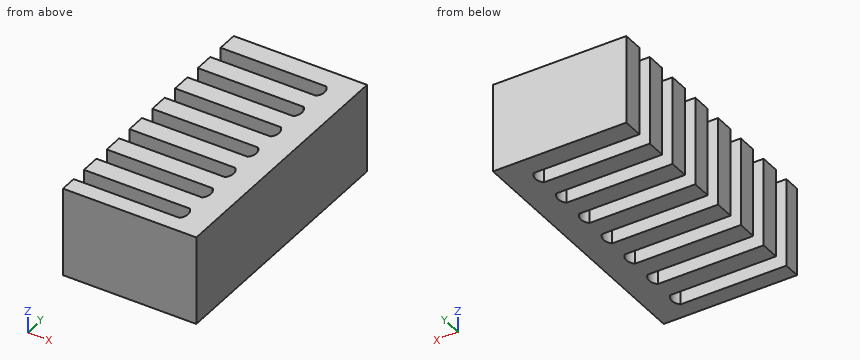
from build123d import *

# Parameters (mm, degrees)
EXTRUDE_1_DEPTH = 5


with BuildPart() as part:
    # 草图1 → 凸台-拉伸1 (new, symmetric)
    with BuildSketch(Plane.XY):
        with BuildLine():
            Line((7.5, -15), (-7.5, -15))
            Line((-7.5, -15), (-7.5, -13.125870379))
            Line((-7.5, -13.125870379), (4.407309833, -13.125870379))
            ThreePointArc((4.407309833, -13.125870379), (4.784555906, -12.215117792), (4.407309833, -11.304365204))
            Line((4.407309833, -11.304365204), (-7.5, -11.304365204))
            Line((-7.5, -11.304365204), (-7.5, -9.125870379))
            Line((-7.5, -9.125870379), (4.407309833, -9.125870379))
            ThreePointArc((4.407309833, -9.125870379), (4.784555906, -8.215117792), (4.407309833, -7.304365204))
            Line((4.407309833, -7.304365204), (-7.5, -7.304365204))
            Line((-7.5, -7.304365204), (-7.5, -5.125870379))
            Line((-7.5, -5.125870379), (4.407309833, -5.125870379))
            ThreePointArc((4.407309833, -5.125870379), (4.784555906, -4.215117792), (4.407309833, -3.304365204))
            Line((4.407309833, -3.304365204), (-7.5, -3.304365204))
            Line((-7.5, -3.304365204), (-7.5, -1.125870379))
            Line((-7.5, -1.125870379), (4.407309833, -1.125870379))
            ThreePointArc((4.407309833, -1.125870379), (4.784555906, -0.215117792), (4.407309833, 0.695634796))
            Line((4.407309833, 0.695634796), (-7.5, 0.695634796))
            Line((-7.5, 0.695634796), (-7.5, 2.874129621))
            Line((-7.5, 2.874129621), (4.407309833, 2.874129621))
            ThreePointArc((4.407309833, 2.874129621), (4.784555906, 3.784882208), (4.407309833, 4.695634796))
            Line((4.407309833, 4.695634796), (-7.5, 4.695634796))
            Line((-7.5, 4.695634796), (-7.5, 6.874129621))
            Line((-7.5, 6.874129621), (4.407309833, 6.874129621))
            ThreePointArc((4.407309833, 6.874129621), (4.784555906, 7.784882208), (4.407309833, 8.695634796))
            Line((4.407309833, 8.695634796), (-7.5, 8.695634796))
            Line((-7.5, 8.695634796), (-7.5, 10.874129621))
            Line((-7.5, 10.874129621), (4.407309833, 10.874129621))
            ThreePointArc((4.407309833, 10.874129621), (4.784555906, 11.784882208), (4.407309833, 12.695634796))
            Line((4.407309833, 12.695634796), (-7.5, 12.695634796))
            Line((-7.5, 12.695634796), (-7.5, 15))
            Line((-7.5, 15), (7.5, 15))
            Line((7.5, 15), (7.5, -15))
        make_face()
    extrude(amount=EXTRUDE_1_DEPTH, both=True)


solid = part.part
Model file for the job. Use its own axes, mm. Coordinates: 2 decimals unless noted, no trailing zeros. Order: outer loops, then holes, each group sorted by start corner. A loop starts at its lowest first (then second) coordinate and runs counter-clockwise, first axis right, second up. Notation, with made-up numbers: M 12,17.25 L 60,17.25 A20 ccw 60,27.25 Z; hole C 48.25,-28.5 d11. An arc over 180 degrees is marked long. Return JSON: item names as keys, results as strings.
1. Drill centre lines: probe 1 along X at (y, z) = (-12.25, -1); probe 2 along X at (y, z) = (-11.75, 4). Where is each one in solid material? Low to high.
Ans:
{"probe 1": "4.78 to 7.5", "probe 2": "4.7 to 7.5"}
2. Saw through at D-D (y = -4.75). Give the cut face in (x, z).
Ans:
{"outline": "M 4.67,-5 L 7.5,-5 L 7.5,5 L 4.67,5 Z"}
3. Saw through at C-C (y = 12.25). Give the cut face in (x, z), and give its area (3 significant figures).
Ans:
{"outline": "M 4.7,-5 L 7.5,-5 L 7.5,5 L 4.7,5 Z", "area": "28.0 mm^2"}
4. Saw through at A-A (x = -6). Give the number of separate pieces and of enclosed holes in the cut face, and give its area (3 significant figures).
Ans:
{"separate pieces": "8", "enclosed holes": "0", "area": "172 mm^2"}
